Verification items for this drawing (mm, ordinates from the low corner). A direction names the side the tool comes from. Round coordinates to 2 decimals unless told otherwise and drop trailing zeros. Write each loop counter-clockwise with the first axis right and the second up, starting at its lowest first coordinate (ties: lowest second). Pieces come first, ordered by that corner, then holes.
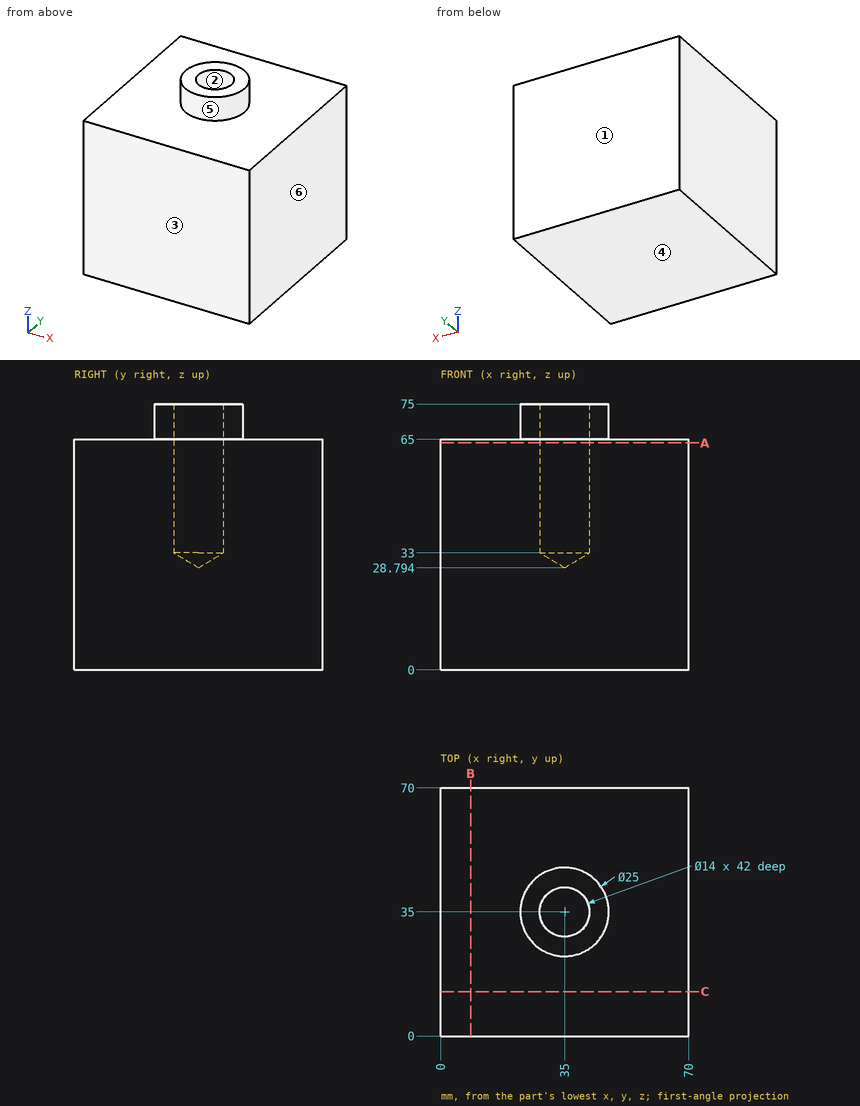
1. Section check B-B (x = 8.5). Record the cut outline in (y, z).
2. Access from +Z, -Z, +X, -X, +Y, -Y to the whole of each face (thin tool, end or side, straight path). Record for the marked faces 5 and 6.
3. Release check for a two-part mould opening along Y. For the marked faces 1, 2, 3 and 4 record: +Y half, -Y half, draft (parallel to the pull), parting line (faces both ways), or undercut.
4. Scan lines: line 1 along X through (y, z) = (35, 64); line 2 along Z through (x, y) = (35.5, 21.5). Record each from-to range of solid material in increasing order.
5. Section check A-A (z = 64). Record the cut outline in (x, y).
6. Depth check by flat-ended pin: pin 1 Ø6 at (y, z) = (39.5, 24.5) entering from -X; pin 2 Ø6 at (x, y) = (10.5, 32) entering from +Z. Enter the tip coordinate at first touch or a pass-through.
Results below:
1. outline: (0, 0) - (70, 0) - (70, 65) - (0, 65) - close
2. face 5: +Z
2. face 6: +Z, -Z, +X, +Y, -Y
3. face 1: +Y half
3. face 2: undercut
3. face 3: -Y half
3. face 4: draft
4. line 1: x = 0 to 28, 42 to 70
4. line 2: z = 0 to 65
5. outline: (0, 0) - (70, 0) - (70, 70) - (0, 70) - close; hole circle Ø14 at (35, 35)
6. pin 1: stops at x = 0
6. pin 2: stops at z = 65
